```python
from build123d import *

# Parameters (mm, degrees)
SKETCH_1_R      = 14.25
SKETCH_1_R_2    = 10
EXTRUDE_1_DEPTH = 0.8
SKETCH_2_R      = 13.5
SKETCH_2_R_2    = 10
EXTRUDE_2_DEPTH = 3.2
FILLET_R0_1_1_R = 0.1


with BuildPart() as part:
    # 草图1 → 凸台-拉伸1 (new body)
    with BuildSketch(Plane(origin=(0, 0, 0), x_dir=(1, 0, 0), z_dir=(0, 1, 0))):
        with Locations(Location((0, 0, 0), (0, 0, 270))):
            Circle(SKETCH_1_R)
        with Locations(Location((0, 0, 0), (0, 0, 270))):
            Circle(SKETCH_1_R_2, mode=Mode.SUBTRACT)
    extrude(amount=EXTRUDE_1_DEPTH)

    # 草图2 → 凸台-拉伸2 (add)
    with BuildSketch(Plane(origin=(0, 0.8, 0), x_dir=(1, 0, 0), z_dir=(0, 1, 0))):
        with Locations(Location((0, 0, 0), (0, 0, 270))):
            Circle(SKETCH_2_R)
        with Locations(Location((0, 0, 0), (0, 0, 270))):
            Circle(SKETCH_2_R_2, mode=Mode.SUBTRACT)
    extrude(amount=EXTRUDE_2_DEPTH)

    # R0.1 圆角1
    fillet_r0_1_1_edges = [part.edges().sort_by_distance(p)[0] for p in [
        (0, 4, -13.5),
        (0, 4, -10),
        (0, 0, -10),
    ]]
    fillet(fillet_r0_1_1_edges, radius=FILLET_R0_1_1_R)


solid = part.part
```
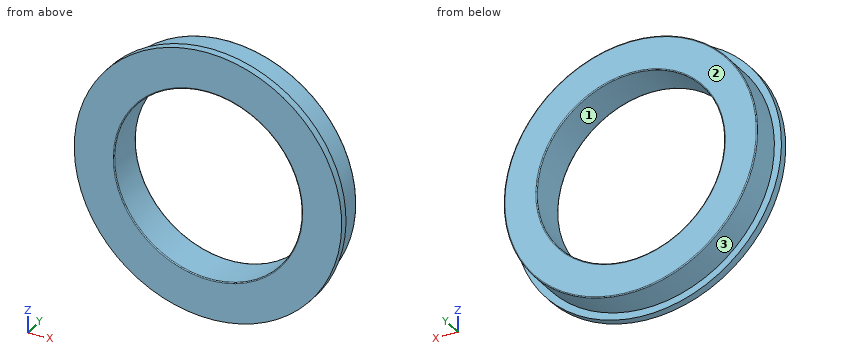
Could you check a few things on this model? Use its own coordinates, in mm. Face numbers are marked on the shaded views. Coordinates: 2 decimals unless noted, no trailing zeros. Write each loop counter-clockwise with the first axis right and the second up, starting at its lowest first coordinate (ties: lowest second). Pieces come first, ordered by that corner, then holes. Notation, with made-up numbers: (63, 69.5) - (122, 69.5) arc R20 ccw to (122, 86.5) - close; hole circle Ø11 at (61, 84). An arc over 180 degrees is marked (long way). Use a Markdown table: item, result.
Q1. Thinking about a two-plate mould opening in Z: for the marked faces 1, 2 and 3, which applies, +Z half, -Z half, draft (parallel to the pull), parting line (faces both ways), or undercut?
Geometry check:
| item | result |
|---|---|
| face 1 | undercut |
| face 2 | draft |
| face 3 | parting line |
Q2. Please list where these lines run through material, in increasing order: L1, parallel to Z at x = 0.25, y = 3.8; L2, parallel to X at y = 0.45, z = -3.5; L3, parallel to X at y = 1.5, z = -1.5.
Geometry check:
| item | result |
|---|---|
| L1 | z = -13.5 to -10, 10 to 13.5 |
| L2 | x = -13.81 to -9.37, 9.37 to 13.81 |
| L3 | x = -13.42 to -9.89, 9.89 to 13.42 |
Q3. Imagine slicing it at C-C (y = 1.8). List the corners of the cut face in (x, z) for me, and give its area (3 significant figures).
Geometry check:
| item | result |
|---|---|
| outline | circle Ø27 at (0, 0); hole circle Ø20 at (0, 0) |
| area | 258 mm2 |
Q4. Imagine slicing it at B-B (z = 0). List the corners of the cut face in (x, y) for me, and give its area (3 significant figures).
Geometry check:
| item | result |
|---|---|
| outline | (-14.25, 0) - (-10.1, 0) arc R0.1 ccw to (-10, 0.1) - (-10, 3.9) arc R0.1 ccw to (-10.1, 4) - (-13.4, 4) arc R0.1 ccw to (-13.5, 3.9) - (-13.5, 0.8) - (-14.25, 0.8) - close; (10, 0.1) arc R0.1 ccw to (10.1, 0) - (14.25, 0) - (14.25, 0.8) - (13.5, 0.8) - (13.5, 3.9) arc R0.1 ccw to (13.4, 4) - (10.1, 4) arc R0.1 ccw to (10, 3.9) - close |
| area | 29.2 mm2 |
Q5. Imagine slicing it at A-A (x = 0). List the corners of the cut face in (y, z) for me.
Geometry check:
| item | result |
|---|---|
| outline | (0, -14.25) - (0.8, -14.25) - (0.8, -13.5) - (3.9, -13.5) arc R0.1 ccw to (4, -13.4) - (4, -10.1) arc R0.1 ccw to (3.9, -10) - (0.1, -10) arc R0.1 ccw to (0, -10.1) - close; (0, 10.1) arc R0.1 ccw to (0.1, 10) - (3.9, 10) arc R0.1 ccw to (4, 10.1) - (4, 13.4) arc R0.1 ccw to (3.9, 13.5) - (0.8, 13.5) - (0.8, 14.25) - (0, 14.25) - close |
Q6. I'm going to push flat-ended pins straight in: pin 1 Ø1.5 at (y, z) = (2, -7) entering from +X; pin 2 Ø16 at (x, z) = (0, 0) entering from +Y. Where does each tip first touch, or does it pass through?
Geometry check:
| item | result |
|---|---|
| pin 1 | stops at x = 11.97 |
| pin 2 | passes through |
